The model under review builds one solid part; all positions refer to its coordinate system, in mm. Face numbers are marked on the shaded views. Give positions to 0.01 mm unless a question says otherwise; leave off trailing zeros. Order: outer loops, then holes, each group sorted by start corner. A loop starts at its lowest first (then second) coordinate and runs counter-clockwise, first axis right, second up. Notation, with made-up numbers: (-10, 66) -> (30, 66) arc R32 cw to (30, 103) -> close; hole circle Ø5 at (7, 82.25). An arc over 180 degrees is marked (long way). Answer as a JSON object with one key per item and string values. Group by question number.
from build123d import *

# Parameters (mm, degrees)
BOSS_EXTRUDE1_START = 7.5
SKETCH1_R           = 225.5
SKETCH1_R_2         = 100
BOSS_EXTRUDE1_DEPTH = 10
SKETCH2_R           = 15
BOSS_EXTRUDE2_DEPTH = 15
SKETCH3_W           = 50
SKETCH3_H           = 48.595629982
CUT_EXTRUDE1_DEPTH  = 321.820043015
SKETCH4_R           = 130
BOSS_EXTRUDE3_DEPTH = 25


with BuildPart() as part:
    # Sketch1 → Boss-Extrude1 (new body)
    with BuildSketch(Plane.XY.offset(BOSS_EXTRUDE1_START)):
        Circle(SKETCH1_R)
        Circle(SKETCH1_R_2, mode=Mode.SUBTRACT)
    extrude(amount=BOSS_EXTRUDE1_DEPTH)


with BuildPart() as body_2:
    # Mirror1: mirrored copy
    add(part.part.mirror(Plane.XY))


with BuildPart() as part_1:
    add(part.part)

    add(body_2.part)  # Boss-Extrude2 merges body 2
    # Sketch2 → Boss-Extrude2 (add)
    with BuildSketch(Plane.XY.offset(-7.5)):
        with Locations((0, 190)):
            Circle(SKETCH2_R)
        with Locations(Location((58.713228931, 180.700738096, 0), (0, 0, 180))):
            Circle(SKETCH2_R)
        with Locations(Location((111.679197936, 153.713228931, 0), (0, 0, 180))):
            Circle(SKETCH2_R)
        with Locations(Location((153.713228931, 111.679197936, 0), (0, 0, 180))):
            Circle(SKETCH2_R)
        with Locations(Location((180.700738096, 58.713228931, 0), (0, 0, 180))):
            Circle(SKETCH2_R)
        with Locations(Location((190, 0, 0), (0, 0, 180))):
            Circle(SKETCH2_R)
        with Locations(Location((180.700738096, -58.713228931, 0), (0, 0, 180))):
            Circle(SKETCH2_R)
        with Locations(Location((153.713228931, -111.679197936, 0), (0, 0, 180))):
            Circle(SKETCH2_R)
        with Locations(Location((111.679197936, -153.713228931, 0), (0, 0, 180))):
            Circle(SKETCH2_R)
        with Locations(Location((58.713228931, -180.700738096, 0), (0, 0, 180))):
            Circle(SKETCH2_R)
        with Locations(Location((0, -190, 0), (0, 0, 180))):
            Circle(SKETCH2_R)
        with Locations(Location((-58.713228931, -180.700738096, 0), (0, 0, 180))):
            Circle(SKETCH2_R)
        with Locations(Location((-111.679197936, -153.713228931, 0), (0, 0, 180))):
            Circle(SKETCH2_R)
        with Locations(Location((-153.713228931, -111.679197936, 0), (0, 0, 180))):
            Circle(SKETCH2_R)
        with Locations(Location((-180.700738096, -58.713228931, 0), (0, 0, 180))):
            Circle(SKETCH2_R)
        with Locations(Location((-190, 0, 0), (0, 0, 180))):
            Circle(SKETCH2_R)
        with Locations(Location((-180.700738096, 58.713228931, 0), (0, 0, 180))):
            Circle(SKETCH2_R)
        with Locations(Location((-153.713228931, 111.679197936, 0), (0, 0, 180))):
            Circle(SKETCH2_R)
        with Locations(Location((-111.679197936, 153.713228931, 0), (0, 0, 180))):
            Circle(SKETCH2_R)
        with Locations(Location((-58.713228931, 180.700738096, 0), (0, 0, 180))):
            Circle(SKETCH2_R)
    extrude(amount=BOSS_EXTRUDE2_DEPTH)

    # Sketch3 → Cut-Extrude1 (cut, through all)
    with BuildSketch(Plane.XY.offset(17.5)):
        with Locations((0, 88.702185009)):
            Rectangle(SKETCH3_W, SKETCH3_H)
    extrude(amount=-CUT_EXTRUDE1_DEPTH, mode=Mode.SUBTRACT)

    # Sketch4 → Boss-Extrude3 (add)
    with BuildSketch(Plane(origin=(0, 0, -17.5), x_dir=(-1, 0, 0), z_dir=(0, 0, -1))):
        Circle(SKETCH4_R)
        with BuildLine():
            Line((-25, 113), (25, 113))
            Line((25, 113), (25, 96.824583655))
            ThreePointArc((25, 96.824583655), (0, -100), (-25, 96.824583655))
            Line((-25, 96.824583655), (-25, 113))
        make_face(mode=Mode.SUBTRACT)
    extrude(amount=BOSS_EXTRUDE3_DEPTH)


solid = part_1.part
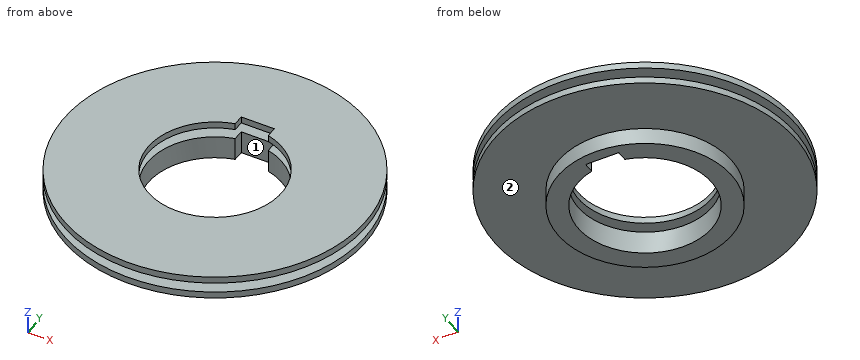
1. For probe 1 along Z at (x, y) = (-126, 103.5); probe 2 along Y at (x, z) = (0, 12.25); probe 3 along Y at (x, z) = (0, -33), list the stretches that pass through material, from the lowest coordinate up. Write a range as [from, to].
2. Take a section at D-D on y = -190. Give the boundary of the cut face in (x, z).
3. Take a section at C-C on z = 2. State how many separate pieces and enclosed holes the cut face has, plus the area to 3 significant figures.
4. Take a section at A-A on x = 0. Give the boundary of the cut face in (y, z), plus the area to 4 significant figures.
5. For pin 1 (10 mm diameter, centred on x = -64.5, z = 7, fed in from +Y); pin 2 (11 mm diameter, centred on y = 108.5, z = 12, fed in from +X); pin 3 (11 mm diameter, centred on y = 106, z = 11.5, fed in from -X), all flat-tipped, find the tip position at first contact; note any pin that passes through.
6. Take a section at B-B on x = -144. Give the boundary of the cut face in (y, z), plus the area to 3 significant figures.
7. Draft analysis for pull direction X (two halves, no side actions). For the marked faces 1 and 2, state which applies: pulls with the +X half, pulls with the -X half, needs draft (parallel to the pull), parting line crosses it, or undercut.
Checks:
{
 "1": {"probe 1": "z = [-17.5, -7.5], [7.5, 17.5]", "probe 2": "y = [-225.5, -100], [113, 225.5]", "probe 3": "y = [-130, -100], [113, 130]"},
 "2": {"outline": "(-121.45, -17.5) -> (121.45, -17.5) -> (121.45, -7.5) -> (70.48, -7.5) -> (70.48, 7.5) -> (121.45, 7.5) -> (121.45, 17.5) -> (-121.45, 17.5) -> (-121.45, 7.5) -> (-70.48, 7.5) -> (-70.48, -7.5) -> (-121.45, -7.5) -> close; hole (-46.94, -7.5) -> (-15, -7.5) -> (-15, 7.5) -> (-46.94, 7.5) -> close; hole (15, -7.5) -> (46.94, -7.5) -> (46.94, 7.5) -> (15, 7.5) -> close"},
 "3": {"separate pieces": "20", "enclosed holes": "0", "area": "14,100 mm2"},
 "4": {"outline": "(-225.5, -17.5) -> (-130, -17.5) -> (-130, -42.5) -> (-100, -42.5) -> (-100, -7.5) -> (-175, -7.5) -> (-175, 7.5) -> (-100, 7.5) -> (-100, 17.5) -> (-225.5, 17.5) -> (-225.5, 7.5) -> (-205, 7.5) -> (-205, -7.5) -> (-225.5, -7.5) -> close; (113, -42.5) -> (130, -42.5) -> (130, -17.5) -> (225.5, -17.5) -> (225.5, -7.5) -> (205, -7.5) -> (205, 7.5) -> (225.5, 7.5) -> (225.5, 17.5) -> (113, 17.5) -> (113, 7.5) -> (175, 7.5) -> (175, -7.5) -> (113, -7.5) -> close", "area": "6,835 mm2"},
 "5": {"pin 1": "stops at y = 217.5", "pin 2": "stops at x = 200.6", "pin 3": "stops at x = -201.87"},
 "6": {"outline": "(-173.53, -17.5) -> (173.53, -17.5) -> (173.53, -7.5) -> (123.11, -7.5) -> (123.11, 7.5) -> (173.53, 7.5) -> (173.53, 17.5) -> (-173.53, 17.5) -> (-173.53, 7.5) -> (-123.11, 7.5) -> (-123.11, -7.5) -> (-173.53, -7.5) -> close; hole (-100.25, -7.5) -> (100.25, -7.5) -> (100.25, 7.5) -> (-100.25, 7.5) -> close", "area": "7,630 mm2"},
 "7": {"face 1": "undercut", "face 2": "needs draft"}
}
